from build123d import *

# Parameters (mm, degrees)
BASE_BLOCK_DEPTH         = 40
TOP_BOSS_PROFILE_W       = 32
TOP_BOSS_PROFILE_H       = 80
TOP_BOSS_PROFILE_R       = 8.381868302
TOP_BOSS_DEPTH           = 21
U_SLOT_W12_DEPTH         = 32
ARM_PROFILE_W            = 50
ARM_PROFILE_H            = 36
ARM_DEPTH                = 84
SQUARE_NOTCH_PROFILE_W   = 20
SQUARE_NOTCH_PROFILE_H   = 36
SQUARE_NOTCH_15X15_DEPTH = 45
ARM_CUT_PROFILE_R        = 10
ARM_CUT_DEPTH            = 36
HOLE_SKETCH_R            = 8.381868302
HOLE_DEPTH               = 125.016127983


with BuildPart() as part:
    # Base Block Profile → Base Block (new, symmetric)
    with BuildSketch(Plane.XY):
        Polygon((0, 0), (0, 36), (34, 61), (66, 61), (66, 0), align=None)
    extrude(amount=BASE_BLOCK_DEPTH, both=True)

    # Top Boss Profile → Top Boss (add)
    with BuildSketch(Plane(origin=(0, 61, 0), x_dir=(1, 0, 0), z_dir=(0, 1, 0))):
        with Locations((50, 0)):
            Rectangle(TOP_BOSS_PROFILE_W, TOP_BOSS_PROFILE_H)
        with Locations(Location((49, 0, 0), (0, 0, 90))):
            Circle(TOP_BOSS_PROFILE_R, mode=Mode.SUBTRACT)
    extrude(amount=TOP_BOSS_DEPTH)

    # U-Slot Profile → U-Slot W12 (cut)
    with BuildSketch(Plane(origin=(66, 0, 0), x_dir=(0, 0, -1), z_dir=(1, 0, 0))):
        Polygon((-40, 82), (-28, 82), (-40, 61), align=None)
        Polygon((40, 61), (28, 82), (40, 82), align=None)
    extrude(amount=-U_SLOT_W12_DEPTH, mode=Mode.SUBTRACT)

    # Arm Profile → Arm (add)
    with BuildSketch(Plane.ZY):
        with Locations((0, 18)):
            Rectangle(ARM_PROFILE_W, ARM_PROFILE_H)
    extrude(amount=ARM_DEPTH)

    # Square Notch Profile → Square Notch 15x15 (cut)
    with BuildSketch(Plane.ZY.offset(84)):
        with Locations((0, 18)):
            Rectangle(SQUARE_NOTCH_PROFILE_W, SQUARE_NOTCH_PROFILE_H)
    extrude(amount=-SQUARE_NOTCH_15X15_DEPTH, mode=Mode.SUBTRACT)

    # Arm Cut Profile → Arm Cut (cut)
    with BuildSketch(Plane(origin=(0, 36, 0), x_dir=(1, 0, 0), z_dir=(0, 1, 0))):
        with Locations((-38.804725968, 0)):
            Circle(ARM_CUT_PROFILE_R)
    extrude(amount=-ARM_CUT_DEPTH, mode=Mode.SUBTRACT)

    # Hole Sketch → Hole (cut, through all)
    with BuildSketch(Plane(origin=(0, 82, 0), x_dir=(1, 0, 0), z_dir=(0, 1, 0))):
        with Locations(Location((49, 0, 0), (0, 0, 90))):
            Circle(HOLE_SKETCH_R)
    extrude(amount=-HOLE_DEPTH, mode=Mode.SUBTRACT)


solid = part.part
Geometry check sheet. Reference: the model listing, model coordinates, mm. A direction names the side the tool comes from. Round coordinates to 2 decimals unless told otherwise and drop trailing zeros. Write each loop counter-clockwise with the first axis right and the second up, starting at its lowest first coordinate (ties: lowest second). Pieces come first, ordered by that corner, then holes.
Item 1: Section check C-C (y = 44). Record the boundary of the cut face in (x, z).
Determined:
outline: (10.88, -40) - (66, -40) - (66, 40) - (10.88, 40) - close; hole circle Ø16.76 at (49, 0)
Item 2: Section check B-B (z = 0). Record the boundary of the cut face in (x, y), plus the area to 3 significant figures.
Determined:
outline: (-28.8, 0) - (40.62, 0) - (40.62, 82) - (34, 82) - (34, 61) - (0, 36) - (-28.8, 36) - close; (57.38, 0) - (66, 0) - (66, 82) - (57.38, 82) - close
area: 3,940 mm2
Item 3: Access from +Z, -Z, +X, -X, +Y, -Y to the whole of each face (thin tool, end or side, straight path). Record for faces 5 (the face through (-41, 18, 25)), 6 (the face through (-84, 18, -18)), 7 (the face through (0, 18, -32)), 8 (the face through (33, 30, -40)), 9 (the face through (-41, 36, -11)).
Determined:
face 5: +Z, -X, +Y, -Y
face 6: +Z, -Z, -X, +Y, -Y
face 7: -Z, -X, +Y, -Y
face 8: -Z, +X, -X, +Y, -Y
face 9: +Z, -Z, -X, +Y
Item 4: Go/stop test with flat-tipped pins: pin 1 Ø12 at (x, z) = (-23.5, -14) entering from +Y; pin 2 Ø4.5 at (y, z) = (15.5, 35.5) entering from -X; pin 3 Ø1.5 at (y, z) = (49, 10) entering from -X. Record where each tip stops, or that it passes through.
Determined:
pin 1: stops at y = 36
pin 2: stops at x = 0
pin 3: stops at x = 16.66
Item 5: Section check A-A (x = 49). Record the boundary of the cut face in (y, z), plus the area to 3 significant figures.
Determined:
outline: (0, -40) - (61, -40) - (82, -28) - (82, -8.38) - (0, -8.38) - close; (0, 8.38) - (82, 8.38) - (82, 28) - (61, 40) - (0, 40) - close
area: 4,930 mm2
Item 6: Mould release check, pull along Z, two halves, no side actions. Record for faces 1 (the face through (-28.807, 18.252, 0.223)), 2 (the face through (-62, 18, 10)), 3 (the face through (50.224, 71.647, 33.916)), 4 (the face through (-84, 18, 17)): +Z half, -Z half, draft (parallel to the pull), parting line (faces both ways), or undercut.
Determined:
face 1: undercut
face 2: undercut
face 3: +Z half
face 4: draft
Item 7: Material ranges on line 1 along X through (y, z) = (69.25, 0); line 2 along X through (y, z) = (25, 0); line 3 along Y through (x, z) = (-11.5, -12), recorded low to high.
Determined:
line 1: x = 34 to 40.62, 57.38 to 66
line 2: x = -28.8 to 40.62, 57.38 to 66
line 3: y = 0 to 36
Item 8: Section check D-D (z = 18.5). Record the boundary of the cut face in (x, y).
Determined:
outline: (-84, 0) - (66, 0) - (66, 82) - (34, 82) - (34, 61) - (0, 36) - (-84, 36) - close
